The listing builds one solid part. Answer for the finished solid, in the listing's coordinates (mm). Face numbers are marked on the shaded views. A direction names the side the tool comes from. Coordinates: 2 decimals unless noted, no trailing zeros. Loops run counter-clockwise (first coordinate to the right, second up) from the corner with the lowest first, then second, coordinate; pieces in that order, holes last. Notation, with made-up numbers: (20, -18) -> (51, -18) arc R21 ccw to (51, 7) -> close; hole circle Ø7 at (-6.5, -4). An arc over 180 degrees is marked (long way). Answer in a Markdown table with one row per item.
```python
from build123d import *

# Parameters (mm, degrees)
SKETCH4_W                                        = 200
SKETCH4_H                                        = 160
SKETCH4_R                                        = 5.5
BOSS_EXTRUDE4_DEPTH                              = 20
HOLE_SIZE_PER_HEX_SOCKET_SCREW_TYPE1_D           = 6.6
HOLE_SIZE_PER_HEX_SOCKET_SCREW_TYPE1_CBORE_D     = 11
HOLE_SIZE_PER_HEX_SOCKET_SCREW_TYPE1_CBORE_DEPTH = 6.8
F_6_0_6_DIAMETER_HOLE1_D                         = 6
SKETCH10_W                                       = 200
SKETCH10_H                                       = 60
CUT_EXTRUDE4_DEPTH                               = 1
CHAMFER1_SIZE                                    = 3


with BuildPart() as part:
    # Sketch4 → Boss-Extrude4 (new body)
    with BuildSketch(Plane(origin=(0, 0, 0), x_dir=(0, 0, -1), z_dir=(1, 0, 0))):
        with Locations((-100, 0)):
            Rectangle(SKETCH4_W, SKETCH4_H)
        with Locations((-125, -65)):
            Circle(SKETCH4_R, mode=Mode.SUBTRACT)
        with Locations((-75, -65)):
            Circle(SKETCH4_R, mode=Mode.SUBTRACT)
        with Locations((-25, -65)):
            Circle(SKETCH4_R, mode=Mode.SUBTRACT)
        with Locations(Location((-125, 65, 0), (0, 0, 180))):
            Circle(SKETCH4_R, mode=Mode.SUBTRACT)
        with Locations(Location((-75, 65, 0), (0, 0, 180))):
            Circle(SKETCH4_R, mode=Mode.SUBTRACT)
        with Locations(Location((-25, 65, 0), (0, 0, 180))):
            Circle(SKETCH4_R, mode=Mode.SUBTRACT)
        with Locations((-175, -65)):
            Circle(SKETCH4_R, mode=Mode.SUBTRACT)
        with Locations((-175, 65)):
            Circle(SKETCH4_R, mode=Mode.SUBTRACT)
        with BuildLine():
            Line((-65, -20), (-115, -20))
            ThreePointArc((-115, -20), (-135, 0), (-115, 20))
            Line((-115, 20), (-65, 20))
            ThreePointArc((-65, 20), (-45, 0), (-65, -20))
        make_face(mode=Mode.SUBTRACT)
    extrude(amount=BOSS_EXTRUDE4_DEPTH)

    # Hole size per hex socket screw type1 (through all)
    with Locations(Plane(origin=(20, 0, 0), x_dir=(0, 0, -1), z_dir=(1, 0, 0))):
        with Locations((-6, 40), (-6, 0), (-6, -40), (-27, -44), (-82, -44), (-137, -44), (-27, 44), (-82, 44), (-137, 44)):
            CounterBoreHole(HOLE_SIZE_PER_HEX_SOCKET_SCREW_TYPE1_D / 2, HOLE_SIZE_PER_HEX_SOCKET_SCREW_TYPE1_CBORE_D / 2, HOLE_SIZE_PER_HEX_SOCKET_SCREW_TYPE1_CBORE_DEPTH)

    # Ø6.0 (6) Diameter Hole1 (through all)
    with Locations(Plane(origin=(20, 0, 0), x_dir=(0, 0, -1), z_dir=(1, 0, 0))):
        with Locations((-6, 25), (-6, -25), (-42, -44), (-122, -44), (-122, 44), (-42, 44)):
            Hole(F_6_0_6_DIAMETER_HOLE1_D / 2)

    # Sketch10 → Cut-Extrude4 (cut)
    with BuildSketch(Plane(origin=(20, 0, 0), x_dir=(0, 0, -1), z_dir=(1, 0, 0))):
        with Locations((-100, 0)):
            Rectangle(SKETCH10_W, SKETCH10_H)
    extrude(amount=-CUT_EXTRUDE4_DEPTH, mode=Mode.SUBTRACT)

    # Chamfer1
    chamfer1_edges = [part.edges().sort_by_distance(p)[0] for p in [
        (10, 80, 200),
        (10, 80, 0),
        (10, -80, 0),
        (10, -80, 200),
    ]]
    chamfer(chamfer1_edges, length=CHAMFER1_SIZE)


solid = part.part
```
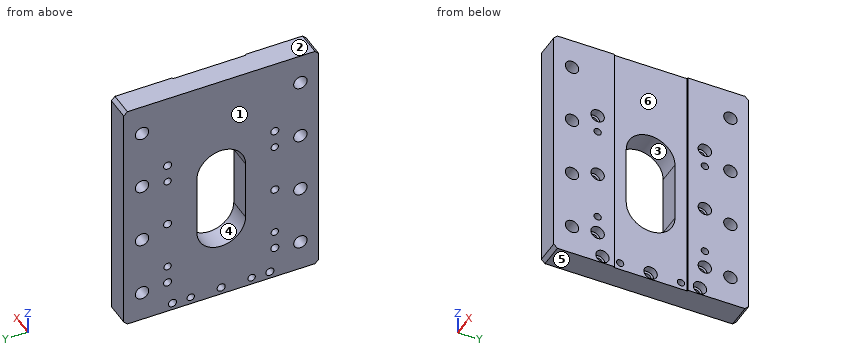
Item 1: Flat-ended cylindrical pins translate along their axes: pin 1 Ø7.5 at (y, z) = (-40, 6) entering from +X; pin 2 Ø12 at (y, z) = (20, 114) entering from +X. Find the tip coordinate at first contact, or state that the pin passes through.
Findings below:
| item | result |
|---|---|
| pin 1 | stops at x = 13.2 |
| pin 2 | stops at x = 19 |
Item 2: Find the intervals of material crossed by probe 1 along Y at (x, z) = (3, 137); probe 2 along Y at (x, z) = (14.75, 6); probe 3 along Y at (x, z) = (7, 6), in increasing order.
Findings below:
| item | result |
|---|---|
| probe 1 | y = -80 to -47.3, -40.7 to 40.7, 47.3 to 80 |
| probe 2 | y = -80 to -45.5, -34.5 to -28, -22 to -5.5, 5.5 to 22, 28 to 34.5, 45.5 to 80 |
| probe 3 | y = -80 to -43.3, -36.7 to -28, -22 to -3.3, 3.3 to 22, 28 to 36.7, 43.3 to 80 |
Item 3: A cutting plane is placed at D-D, the plane z = 122. Determine the outline of the cut face in (x, y) (3 decimals), plus the area to 3 significant figures.
Findings below:
| item | result |
|---|---|
| outline | (0, -80) -> (20, -80) -> (20, -69.61) -> (0, -69.61) -> close; (0, -60.39) -> (20, -60.39) -> (20, -47) -> (0, -47) -> close; (0, -41) -> (20, -41) -> (20, -30) -> (19, -30) -> (19, -18.735) -> (0, -18.735) -> close; (0, 18.735) -> (19, 18.735) -> (19, 30) -> (20, 30) -> (20, 41) -> (0, 41) -> close; (0, 47) -> (20, 47) -> (20, 60.39) -> (0, 60.39) -> close; (0, 69.61) -> (20, 69.61) -> (20, 80) -> (0, 80) -> close |
| area | 1,820 mm2 |
Item 4: Determine the mould class of the marked faces 1, 2 and 3 for opening direction Z: +Z half, -Z half, draft (parallel to the pull), parting line (faces both ways), or undercut.
Findings below:
| item | result |
|---|---|
| face 1 | draft |
| face 2 | +Z half |
| face 3 | undercut |
Item 5: A cutting plane is placed at B-B, the plane z = 102. Determine the outline of the cut face in (x, y), plus the area to 3 significant figures.
Findings below:
| item | result |
|---|---|
| outline | (0, -80) -> (20, -80) -> (20, -30) -> (19, -30) -> (19, -20) -> (0, -20) -> close; (0, 20) -> (19, 20) -> (19, 30) -> (20, 30) -> (20, 80) -> (0, 80) -> close |
| area | 2,380 mm2 |
Item 6: A tool of negligible diameter and unlimited length cuts with its end or side. For the marked faces 4, 5 and 6, from which of +Z, -Z, +X, -X, +Y, -Y can it reach the whole face along a straight path? Write none if from no direction.
Findings below:
| item | result |
|---|---|
| face 4 | +X, -X |
| face 5 | -Z, +X, -X, +Y, -Y |
| face 6 | +Z, -Z, +X |
Item 7: A cutting plane is placed at A-A, the plane y = 0. Determine the outline of the cut face in (x, z).
Findings below:
| item | result |
|---|---|
| outline | (0, 0) -> (19, 0) -> (19, 0.5) -> (13.2, 0.5) -> (13.2, 2.7) -> (0, 2.7) -> close; (0, 9.3) -> (13.2, 9.3) -> (13.2, 11.5) -> (19, 11.5) -> (19, 45) -> (0, 45) -> close; (0, 135) -> (19, 135) -> (19, 200) -> (0, 200) -> close |
Item 8: A cutting plane is placed at C-C, the plane z = 27. Count the separate pieces of the cut face and the enclosed holes in it, plus the area to 3 significant figures.
Findings below:
| item | result |
|---|---|
| separate pieces | 5 |
| enclosed holes | 0 |
| area | 2,410 mm2 |
